Geometry: final body of the model. Coordinates: model frame, mm. A direction names the side the tool comes from. Give positions to 0.01 mm unless a question says otherwise; leave off trailing zeros. Write each loop counter-clockwise with the first axis right and the second up, starting at its lowest first coordinate (ties: lowest second). Pieces come first, ordered by that corner, then holes. Notation, with made-up numbers: M -16,-25.5 L -1,-25.5 A27 cw -1,0.5 Z; hole C 88,56.5 d2. An arc over 180 degrees is marked long. Answer as a JSON object with one key per item and string values.
from build123d import *

# Parameters (mm, degrees)
BOSS_EXTRUDE1_DEPTH   = 12.5
SKETCH3_R             = 8.7
BOSS_EXTRUDE2_DEPTH   = 125
BOSS_EXTRUDE3_DEPTH   = 9.5
HOLE1_D               = 4.134
HOLE1_DEPTH           = 5
HOLE1_CSINK_D         = 5
HOLE1_CSINK_ANGLE     = 90
HOLE1_TIP             = 1.193383006
HOLE2_D               = 4.134
HOLE2_DEPTH           = 5
HOLE2_CSINK_D         = 5
HOLE2_CSINK_ANGLE     = 90
HOLE2_TIP             = 1.193383006
BOSS_EXTRUDE4_DEPTH   = 138
LINEAR_PATTERN1_COUNT = 2
LINEAR_PATTERN1_PITCH = 132


with BuildPart() as part:
    # Sketch1 → Revolve1 (revolve)
    with BuildSketch(Plane.XY, mode=Mode.PRIVATE) as revolve1_sk:
        Polygon((-8, 0), (-8, 4.3865), (-7.3865, 5), (0, 5), (0, 0), align=None)
    revolve(revolve1_sk.sketch.rotate(Axis((0, 0, 0), (-1, 0, 0)), 270), axis=Axis((0, 0, 0), (-1, 0, 0)))

    # Sketch2 → Boss-Extrude1 (add)
    with BuildSketch(Plane(origin=(0, 0, 0), x_dir=(0, 0, -1), z_dir=(1, 0, 0))):
        with BuildLine():
            Line((-4.034538387, -9.15), (4.034538387, -9.15))
            ThreePointArc((4.034538387, -9.15), (7.071067812, -7.071067812), (9.15, -4.034538387))
            Line((9.15, -4.034538387), (9.15, 4.034538387))
            ThreePointArc((9.15, 4.034538387), (7.071067812, 7.071067812), (4.034538387, 9.15))
            Line((4.034538387, 9.15), (-4.034538387, 9.15))
            ThreePointArc((-4.034538387, 9.15), (-7.071067812, 7.071067812), (-9.15, 4.034538387))
            Line((-9.15, 4.034538387), (-9.15, -4.034538387))
            ThreePointArc((-9.15, -4.034538387), (-7.071067812, -7.071067812), (-4.034538387, -9.15))
        make_face()
    extrude(amount=BOSS_EXTRUDE1_DEPTH)

    # Sketch3 → Boss-Extrude2 (add)
    with BuildSketch(Plane(origin=(12.5, 0, 0), x_dir=(0, 0, -1), z_dir=(1, 0, 0))):
        Circle(SKETCH3_R)
    extrude(amount=BOSS_EXTRUDE2_DEPTH)

    # Sketch4 → Boss-Extrude3 (add)
    with BuildSketch(Plane(origin=(137.5, 0, 0), x_dir=(0, 0, -1), z_dir=(1, 0, 0))):
        with BuildLine():
            Line((-4.034538387, -9.15), (4.034538387, -9.15))
            ThreePointArc((4.034538387, -9.15), (7.071067812, -7.071067812), (9.15, -4.034538387))
            Line((9.15, -4.034538387), (9.15, 4.034538387))
            ThreePointArc((9.15, 4.034538387), (7.071067812, 7.071067812), (4.034538387, 9.15))
            Line((4.034538387, 9.15), (-4.034538387, 9.15))
            ThreePointArc((-4.034538387, 9.15), (-7.071067812, 7.071067812), (-9.15, 4.034538387))
            Line((-9.15, 4.034538387), (-9.15, -4.034538387))
            ThreePointArc((-9.15, -4.034538387), (-7.071067812, -7.071067812), (-4.034538387, -9.15))
        make_face()
    extrude(amount=BOSS_EXTRUDE3_DEPTH)

    # Hole1
    with Locations(Plane(origin=(0, 9.15, 0), x_dir=(1, 0, 0), z_dir=(0, 1, 0))):
        with Locations((8, 0)):
            CounterSinkHole(HOLE1_D / 2, HOLE1_CSINK_D / 2, depth=HOLE1_DEPTH, counter_sink_angle=HOLE1_CSINK_ANGLE)
            with Locations((0, 0, -(HOLE1_DEPTH + HOLE1_TIP / 2))):  # 120° drill point
                Cone(0, HOLE1_D / 2, HOLE1_TIP, mode=Mode.SUBTRACT)

    # Hole2
    with Locations(Plane(origin=(0, 9.15, 0), x_dir=(1, 0, 0), z_dir=(0, 1, 0))):
        with Locations((142, 0)):
            CounterSinkHole(HOLE2_D / 2, HOLE2_CSINK_D / 2, depth=HOLE2_DEPTH, counter_sink_angle=HOLE2_CSINK_ANGLE)
            with Locations((0, 0, -(HOLE2_DEPTH + HOLE2_TIP / 2))):  # 120° drill point
                Cone(0, HOLE2_D / 2, HOLE2_TIP, mode=Mode.SUBTRACT)

    # Sketch9 → Cut-Revolve1 (revolve, cut)
    with BuildSketch(Plane.XY, mode=Mode.PRIVATE) as cut_revolve1_sk:
        Polygon((-8, 0), (-8, 2.5), (12.5, 2.5), (12.5, 8), (117.5, 8), (117.5, 0), align=None)
    revolve(cut_revolve1_sk.sketch.rotate(Axis((50, 0, 0), (-1, 0, 0)), 270), axis=Axis((50, 0, 0), (-1, 0, 0)), mode=Mode.SUBTRACT)

    # Sketch10 → Boss-Extrude4 (add)
    with BuildSketch(Plane(origin=(6, 0, 0), x_dir=(0, 0, -1), z_dir=(1, 0, 0))):
        Polygon((-4, -9.15), (-4, -14.15), (-1.65, -14.15), (-1.65, -12.95), (-2.8, -12.95), (-2.8, -10.35), (2.8, -10.35), (2.8, -12.95), (1.65, -12.95), (1.65, -14.15), (4, -14.15), (4, -9.15), align=None)
    extrude(amount=BOSS_EXTRUDE4_DEPTH)

    # Sketch11 → Revolve2 (revolve)
    with BuildSketch(Plane.XY):
        with BuildLine():
            Line((6.249727286, -10.35), (9, -10.35))
            Line((9, -10.35), (9, -12.35))
            ThreePointArc((9, -12.35), (7.299705908, -11.797136224), (6.249727286, -10.35))
        make_face()
    revolve2 = revolve(axis=Axis((9, 50, 0), (0, -1, 0)))

    # Linear pattern1: Revolve2 ×2
    with Locations(*[(i * LINEAR_PATTERN1_PITCH, 0, 0) for i in range(1, LINEAR_PATTERN1_COUNT)]):
        add(revolve2)


solid = part.part
1) Line query: line 1 (Y direction, x = 85.5, z = 0); line 2 (X direction, y = 5.25, z = -3); line 3 (Z direction, x = 34, y = -10.75). Output: solid intervals per line, ascending. Write a range as from..to.
Geometry check:
{"line 1": "y = -10.35..-9.15, -8.7..-8, 8..8.7", "line 2": "x = 0..12.5, 117.5..147", "line 3": "z = -4..-2.8, 2.8..4"}
2) Cut plane B-B on y = 0. Return loops of the section in (x, z), and give its area (3 significant figures).
Geometry check:
{"outline": "M -8,-4.39 L -7.39,-5 L 0,-5 L 0,-9.15 L 12.5,-9.15 L 12.5,-8.7 L 137.5,-8.7 L 137.5,-9.15 L 147,-9.15 L 147,9.15 L 137.5,9.15 L 137.5,8.7 L 12.5,8.7 L 12.5,9.15 L 0,9.15 L 0,5 L -7.39,5 L -8,4.39 L -8,2.5 L 12.5,2.5 L 12.5,8 L 117.5,8 L 117.5,-8 L 12.5,-8 L 12.5,-2.5 L -8,-2.5 Z", "area": "875 mm2"}
3) Cut plane A-A on x = 37. Return loops of the section in (y, z), and give its area (3 significant figures).
Geometry check:
{"outline": "M -14.15,-4 L -9.15,-4 L -9.15,4 L -14.15,4 L -14.15,1.65 L -12.95,1.65 L -12.95,2.8 L -10.35,2.8 L -10.35,-2.8 L -12.95,-2.8 L -12.95,-1.65 L -14.15,-1.65 Z; C 0,0 d17.4; hole C 0,0 d16", "area": "58.2 mm2"}
4) Contact query for flat-ended pins moving along their axis: P1, Ø4, axis at x = 85.5, z = -2, coming from the +Y side; P2, Ø1, axis at x = 35.5, z = -5.5, coming from the +Y side; P3, Ø1, axis at x = 62, z = 4.5, coming from the +Y side. Output: stop coordinate, or through.
Geometry check:
{"P1": "stops at y = 8.7", "P2": "stops at y = 7.12", "P3": "stops at y = 7.73"}
5) Pull-direction query (X, two-part tool) for faces 4 (the flat face through (-8, -2, -2)), 5 (the cylindrical face through (10.065, 6.402, -0.091)), 6 (the flat face through (142, 0, 9.15)); classes: pulls with the +X half, pulls with the -X half, needs draft (parallel to the pull), parting line crosses it, or undercut.
Geometry check:
{"face 4": "pulls with the -X half", "face 5": "undercut", "face 6": "needs draft"}
6) Set-up query: faces 1 (the cylindrical face through (142.18, 7.03, -7.11)), 2 (the flat face through (12.5, 2, -2)), 3 (the flat face through (6, -10, 0)). Return all of +Z, -Z, +X, -X, +Y, -Y with unobstructed straight access to the full face (end or side cutting, diameter ignored); none if empty.
Geometry check:
{"face 1": "-Z, +X, -X, +Y", "face 2": "none", "face 3": "+Z, -Z, -X, -Y"}
